Input: part model. Units: mm. Frame: model coordinates. A direction names the side the tool comes from. Give positions to 0.01 mm unless a question says otherwise; leave off trailing zeros. Write each loop counter-clockwise with the first axis right and the second up, starting at its lowest first coordinate (ties: lowest second). Pieces come first, ordered by that corner, then holes.
```python
from build123d import *

# Parameters (mm, degrees)
SKETCH_1_W                = 95
SKETCH_1_H                = 100
EXTRUDE_1_DEPTH           = 12
SKETCH_9_W                = 15.5
SKETCH_9_H                = 88
CUT_EXTRUDE_4_DEPTH       = 139.452157802
HOLE_WIZARD_6_5_6_5_1_D   = 6.5
SKETCH_12_R               = 17.5
CUT_EXTRUDE_5_DEPTH       = 139.452157802
FILLET_1_R                = 10
HOLE_WIZARD_5_0_5_1_D     = 5
HOLE_WIZARD_5_0_5_1_DEPTH = 10
HOLE_WIZARD_5_0_5_1_TIP   = 1.502151548
FILLET_2_R                = 2
MM_1_D                    = 9
HOLE_WIZARD_M6_1_D        = 5
HOLE_WIZARD_M6_2_D        = 5


with BuildPart() as part:
    # 草图1 → 凸台-拉伸1 (new body)
    with BuildSketch(Plane(origin=(0, 0, 0), x_dir=(1, 0, 0), z_dir=(0, 1, 0))):
        with Locations((47.5, -50)):
            Rectangle(SKETCH_1_W, SKETCH_1_H)
    extrude(amount=EXTRUDE_1_DEPTH)

    # 草图9 → 切除-拉伸4 (cut, through all)
    with BuildSketch(Plane(origin=(0, 12, 0), x_dir=(1, 0, 0), z_dir=(0, 1, 0))):
        with Locations((7.75, -56)):
            Rectangle(SKETCH_9_W, SKETCH_9_H)
        with Locations((87.25, -56)):
            Rectangle(SKETCH_9_W, SKETCH_9_H)
    extrude(amount=-CUT_EXTRUDE_4_DEPTH, mode=Mode.SUBTRACT)

    # Ø6.5 (6.5) 直径孔1 (through all)
    with Locations(Plane.XY.offset(12)):
        with Locations((6, 6), (89, 6)):
            Hole(HOLE_WIZARD_6_5_6_5_1_D / 2)

    # 草图12 → 切除-拉伸5 (cut, through all)
    with BuildSketch(Plane(origin=(0, 12, 0), x_dir=(1, 0, 0), z_dir=(0, 1, 0))):
        with Locations(Location((47.5, -68, 0), (0, 0, 270))):
            Circle(SKETCH_12_R)
    extrude(amount=-CUT_EXTRUDE_5_DEPTH, mode=Mode.SUBTRACT)

    # 圆角1
    fillet_1_edges = [part.edges().sort_by_distance(p)[0] for p in [
        (15.5, 6, 100),
        (79.5, 6, 100),
    ]]
    fillet(fillet_1_edges, radius=FILLET_1_R)

    # Ø5.0 (5) 直径孔1
    with Locations(Plane(origin=(0, 0, 0), x_dir=(-1, 0, 0), z_dir=(0, 0, -1))):
        with Locations((-67.5, 6), (-27.5, 6)):
            Hole(HOLE_WIZARD_5_0_5_1_D / 2, depth=HOLE_WIZARD_5_0_5_1_DEPTH)
            with Locations((0, 0, -(HOLE_WIZARD_5_0_5_1_DEPTH + HOLE_WIZARD_5_0_5_1_TIP / 2))):  # 118° drill point
                Cone(0, HOLE_WIZARD_5_0_5_1_D / 2, HOLE_WIZARD_5_0_5_1_TIP, mode=Mode.SUBTRACT)

    # 圆角2
    fillet_2_edges = [part.edges().sort_by_distance(p)[0] for p in [
        (15.5, 6, 12),
        (79.5, 6, 12),
    ]]
    fillet(fillet_2_edges, radius=FILLET_2_R)

    # 大小mm 暗销孔1 (through all)
    with Locations(Plane(origin=(0, 0, 0), x_dir=(-1, 0, 0), z_dir=(0, -1, 0))):
        with Locations((-72.5, -43), (-72.5, -93), (-22.5, -93), (-22.5, -43)):
            Hole(MM_1_D / 2)

    # M6 螺纹孔1 (through all)
    with Locations(Plane(origin=(0, 0, 0), x_dir=(-1, 0, 0), z_dir=(0, -1, 0))):
        with Locations((-47.5, -44.5)):
            Hole(HOLE_WIZARD_M6_1_D / 2)

    # M6 螺纹孔2 (through all)
    with Locations(Plane(origin=(0, 0, 0), x_dir=(-1, 0, 0), z_dir=(0, -1, 0))):
        with Locations((-47.5, -18.5)):
            Hole(HOLE_WIZARD_M6_2_D / 2)


solid = part.part
```
Q1. Access query for faces 1 (the cylindrical face through (26, 8, 5)), 2 (the flat face through (10, 6, 12)), 3 (the flat face through (85, 6, 12)). Directions: +Z, -Z, +X, -X, +Y, -Y. A direction counts if a zero-diameter tool reaches every point of the face in a straight line with its end or side. Return the directions, or none.
Q2. Pin query (flat end, axial travel): pin 1 (3 mm diameter, centred on x = 47.5, z = 44.5, fed in from -Y); pin 2 (2 mm diameter, centred on y = 9.5, z = 71.5, fed in from -X). Return the tip coordinate at first contact, or that it passes through.
Q3. Section D-D, the plane z = 93. Return the cut outline in (x, y), then the cut area to 3 significant figures.
Q4. Section C-C, the plane y = 1.25. Return the cut outline in (x, z), then the cut area to 3 significant figures.
Q5. Material intervals for line 1 along Y through (x, z) = (89, 8); line 2 along Y through (x, z) = (27.5, 2); line 3 along X through (y, z) = (8.25, 6), sorted ascending.
Q6. Section A-A, the plane x = 89. Return the cut outline in (y, z), then the cut area to 3 significant figures.
Q7. Mould query, pull axis Z, two halves, no side actions, for faces 4 (the cylindrical face through (18.35, 5.92, 96.99)), 5 (the cylindrical face through (64.85, 6.08, 65.72)), 6 (the cylindrical face through (21.91, 6.08, 88.54)), 7 (the cylindrical face through (69.885, 6.751, 5.07)). Classes: +Z half, -Z half, draft (parallel to the pull), parting line (faces both ways), or undercut.
Q8. Section B-B, the plane z = 68. Return the cut outline in (x, y), then the cut area to 3 significant figures.
Solutions:
1. face 1: -Z
1. face 2: +Z, -X, +Y, -Y
1. face 3: +Z, +X, +Y, -Y
2. pin 1: passes through
2. pin 2: stops at x = 15.5
3. outline: (15.96, 0) - (18, 0) - (18, 12) - (15.96, 12) - close; (27, 0) - (68, 0) - (68, 12) - (27, 12) - close; (77, 0) - (79.04, 0) - (79.04, 12) - (77, 12) - close
3. area: 541 mm2
4. outline: (0, 0) - (95, 0) - (95, 12) - (81.5, 12) arc R2 cw to (79.5, 14) - (79.5, 90) arc R10 ccw to (69.5, 100) - (25.5, 100) arc R10 ccw to (15.5, 90) - (15.5, 14) arc R2 cw to (13.5, 12) - (0, 12) - close; hole circle Ø9 at (22.5, 43); hole circle Ø9 at (22.5, 93); hole circle Ø35 at (47.5, 68); hole circle Ø5 at (47.5, 18.5); hole circle Ø5 at (47.5, 44.5); hole circle Ø9 at (72.5, 43); hole circle Ø9 at (72.5, 93)
4. area: 5,470 mm2
5. line 1: y = 0 to 2.75, 9.25 to 12
5. line 2: y = 0 to 3.5, 8.5 to 12
5. line 3: x = 0 to 3.65, 8.35 to 26.41, 28.59 to 66.41, 68.59 to 86.65, 91.35 to 95
6. outline: (0, 0) - (2.75, 0) - (2.75, 12) - (0, 12) - close; (9.25, 0) - (12, 0) - (12, 12) - (9.25, 12) - close
6. area: 66.0 mm2
7. face 4: +Z half
7. face 5: undercut
7. face 6: undercut
7. face 7: draft
8. outline: (15.5, 0) - (30, 0) - (30, 12) - (15.5, 12) - close; (65, 0) - (79.5, 0) - (79.5, 12) - (65, 12) - close
8. area: 348 mm2
